Here's how the part is built. I have some questions about the finished solid (model axes, mm). Face numbers are marked on the shaded views. Give positions to 0.01 mm unless a question says otherwise; leave off trailing zeros. Loops run counter-clockwise (first coordinate to the right, second up) from the corner with the lowest first, then second, coordinate; pieces in that order, holes last. Notation, with made-up numbers: M 5,14.5 L 14,14.5 A19 ccw 14,42.5 Z; hole C 66.25,-30 d3. An arc over 180 degrees is marked long. Answer as CSV lines item,"result". Start each with the question number.
Item 1: I want a section at C-C on y = 0. List the corners of the cut face in (x, z) for me, plus the area to 3 significant figures.
Item 2: Will these pins go through, and if not, where does the flat tip stop? P1, Ø2, axis at y = -10.5, z = 9.5, coming from the +X side; P2, Ø1.5, axis at y = 8.5, z = 2.5, coming from the +X side; P3, Ø2, axis at x = -7, y = -11.5, coming from the +Z side; P4, Ø1, axis at x = -2, z = 8.5, coming from the -Y side.
Item 3: I want a section at A-A on z = 8.75. List the corners of the cut face in (x, y) for me, plus the area to 3 significant figures.
Item 4: If we mould it in two halves opening along Y, with no side actions, what happens to the marked faces 1, 2 and 3? For each: released by +Y, released by -Y, zero draft, split by the parting line, or undercut.
Item 5: If I drill on line 1 along X through (y, z) = (6, 12.5); line 2 along Y through (x, z) = (0, 11.5); line 3 along Y through (x, z) = (9.5, 7), over which ranges is the centre line in solid material (lowest first)? Write a range as from..to.
Item 6: I want a section at B-B on x = -5. List the corners of the cut face in (y, z) for me, plus the area to 3 significant figures.
Item 7: I want a section at D-D on x = 17. List the corners of the cut face in (y, z) for me.
from build123d import *

# Parameters (mm, degrees)
SKETCH1_R           = 15
BOSS_EXTRUDE1_DEPTH = 15


with BuildPart() as part:
    # Sketch1 → Boss-Extrude1 (new body)
    with BuildSketch(Plane.XY):
        Polygon((9.932712467, 18.912285858), (-11.412163764, 18.058124254), (-21.34487623, -0.854161605), (-9.932712467, -18.912285858), (11.412163764, -18.058124254), (21.34487623, 0.854161605), align=None)
        Circle(SKETCH1_R, mode=Mode.SUBTRACT)
    extrude(amount=BOSS_EXTRUDE1_DEPTH)


solid = part.part
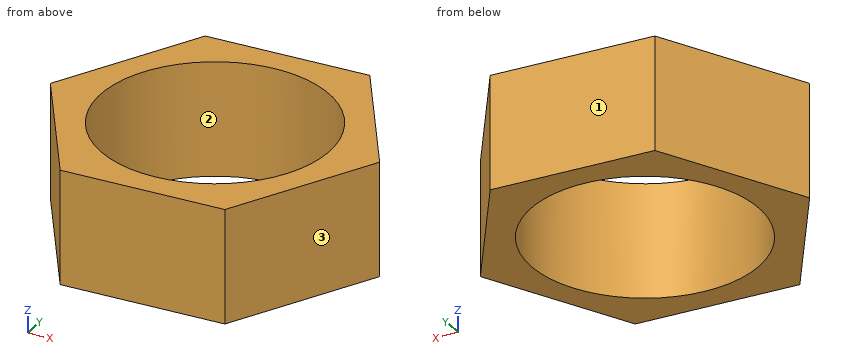
Result:
1,outline,"M -20.9,0 L -15,0 L -15,15 L -20.9,15 Z; M 15,0 L 20.9,0 L 20.9,15 L 15,15 Z"
1,area,"177 mm^2"
2,P1,"x = 15.91"
2,P2,"x = 16.99"
2,P3,"through"
2,P4,"y = -18.61"
3,outline,"M -21.34,-0.85 L -9.93,-18.91 L 11.41,-18.06 L 21.34,0.85 L 9.93,18.91 L -11.41,18.06 Z; hole C 0,0 d30"
3,area,"479 mm^2"
4,face 1,"released by +Y"
4,face 2,"undercut"
4,face 3,"released by -Y"
5,line 1,"-17.75..-13.75, 13.75..18.09"
5,line 2,"-18.51..-15, 15..18.51"
5,line 3,"-18.13..-11.61, 11.61..18.89"
6,outline,"M -18.71,0 L -14.14,0 L -14.14,15 L -18.71,15 Z; M 14.14,0 L 18.31,0 L 18.31,15 L 14.14,15 Z"
6,area,"131 mm^2"
7,outline,"M -7.42,0 L 7.73,0 L 7.73,15 L -7.42,15 Z"
